Could you check a few things on this model? Use its own coordinates, in mm. Face numbers are marked on the shaded views. A direction names the side the tool comes from. Coordinates: 2 decimals unless noted, no trailing zeros. Loops run counter-clockwise (first coordinate to the right, second up) from the corner with the lowest first, then second, coordinate; pieces in that order, holes last. Notation, with made-up numbers: (-9, 20) -> (37, 20) arc R32 cw to (37, 52) -> close; hole circle Ø4 at (0, -17). An arc over 180 degrees is marked (long way). One line per question, with ' | ' between items.
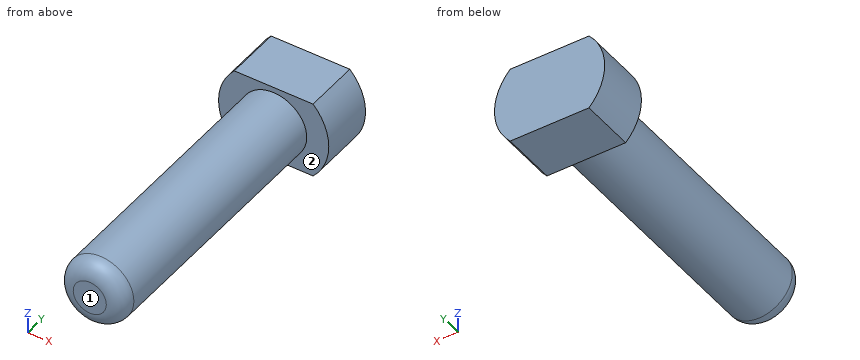
```python
from build123d import *

# Parameters (mm, degrees)
SKETCH_1_R          = 10
EXTRUDE_1_DEPTH     = 30
CUT_EXTRUDE_START   = -50
SKETCH_2_R          = 10
SKETCH_2_R_2        = 6
CUT_EXTRUDE_1_DEPTH = 50
FILLET_1_R          = 3
CUT_EXTRUDE_3_DEPTH = 10


with BuildPart() as part:
    # 草图1 → 凸台-拉伸1 (new, symmetric)
    with BuildSketch(Plane(origin=(0, 0, 0), x_dir=(1, 0, 0), z_dir=(0, 1, 0))):
        with Locations(Location((0, 0, 0), (0, 0, 270))):
            Circle(SKETCH_1_R)
    extrude(amount=EXTRUDE_1_DEPTH, both=True)

    # 草图2 → 切除-拉伸1 (cut)
    with BuildSketch(Plane.XZ.offset(30).offset(CUT_EXTRUDE_START)):
        with Locations(Location((0, 0, 0), (0, 0, 270))):
            Circle(SKETCH_2_R)
        with Locations(Location((0, 0, 0), (0, 0, 270))):
            Circle(SKETCH_2_R_2, mode=Mode.SUBTRACT)
    extrude(amount=CUT_EXTRUDE_1_DEPTH, mode=Mode.SUBTRACT)

    # 圆角1
    fillet_1_edges = [part.edges().sort_by_distance(p)[0] for p in [
        (0, -30, 6),
    ]]
    fillet(fillet_1_edges, radius=FILLET_1_R)

    # 草图3 → 切除-拉伸3 (cut)
    with BuildSketch(Plane(origin=(0, 30, 0), x_dir=(1, 0, 0), z_dir=(0, 1, 0))):
        with BuildLine():
            Line((-7.141428429, 7), (7.141428429, 7))
            ThreePointArc((7.141428429, 7), (0, 10), (-7.141428429, 7))
        make_face()
        with BuildLine():
            Line((-7.141428429, -7), (7.141428429, -7))
            ThreePointArc((7.141428429, -7), (0, -10), (-7.141428429, -7))
        make_face()
    extrude(amount=-CUT_EXTRUDE_3_DEPTH, mode=Mode.SUBTRACT)


solid = part.part
```
Q1. Imagine slicing it at A-A on y = -3. Write out the boundary of the cut face in (x, z), plus the area to 3 significant figures.
Values follow:
outline: circle Ø12 at (0, 0) | area: 113 mm2
Q2. Imagine slicing it at B-B on y = 23.5. Write out the boundary of the cut face in (x, z), plus the area to 3 significant figures.
Values follow:
outline: (-7.14, -7) -> (7.14, -7) arc R10 ccw to (7.14, 7) -> (-7.14, 7) arc R10 ccw to start | area: 255 mm2
Q3. For the marked faces 1 and 2, which set-ups out of +Z, -Z, +X, -X, +Y, -Y let a thin tool reach every point of the face, with its end or its side?
Values follow:
face 1: +Z, -Z, +X, -X, -Y | face 2: -Y
Q4. For pin 1 (2 mm diameter, centred on x = 2, y = -3, fed in from +Z); pin 2 (10 mm diameter, centred on x = 5, y = -10, fed in from +Z); pin 3 (1.5 mm diameter, centred on y = -3.5, z = 2.5, fed in from -X), each with a flat end and sliding along its axis, tell me the tip position at first contact or that it passes through.
Values follow:
pin 1: stops at z = 5.92 | pin 2: stops at z = 6 | pin 3: stops at x = -5.74
Q5. Please list where these lines run through material, in increasing order: L1, parallel to Y at x = -8, z = -4.75; L2, parallel to X at y = 9, z = -1.25; L3, parallel to X at y = 28.5, z = 3. Write a range as [from, to].
Values follow:
L1: y = [20, 30] | L2: x = [-5.87, 5.87] | L3: x = [-9.54, 9.54]
